The listing builds one solid part. Answer for the finished solid, in the listing's coordinates (mm). Face numbers are marked on the shaded views. A direction names the side the tool comes from. Round coordinates to 2 decimals unless told otherwise and drop trailing zeros. Order: outer loops, then holes, each group sorted by start corner. A loop starts at its lowest first (then second) coordinate and runs counter-clockwise, first axis right, second up. Notation, with made-up numbers: (72, -6.5) - (100, -6.5) arc R24 cw to (100, 13.5) - close; hole circle Ø8 at (33, -25.5). An arc over 180 degrees is marked (long way). Write item = value, one per line.
from build123d import *

# Parameters (mm, degrees)
SKETCH1_R           = 5
BOSS_EXTRUDE1_DEPTH = 25
SKETCH2_R           = 4
BOSS_EXTRUDE2_DEPTH = 20
SKETCH3_OUTSIDE_W   = 21.434
SKETCH3_OUTSIDE_H   = 21.434
SKETCH3_OUTSIDE_R   = 3
CUT_EXTRUDE1_DEPTH  = 2


with BuildPart() as part:
    # Sketch1 → Boss-Extrude1 (new body)
    with BuildSketch(Plane.XY):
        Circle(SKETCH1_R)
    extrude(amount=BOSS_EXTRUDE1_DEPTH)

    # Sketch2 → Boss-Extrude2 (add)
    with BuildSketch(Plane.XY.offset(25)):
        Circle(SKETCH2_R)
    extrude(amount=BOSS_EXTRUDE2_DEPTH)

    # Sketch3 outside → Cut-Extrude1 (cut)
    with BuildSketch(Plane.XY.offset(25)):
        Rectangle(SKETCH3_OUTSIDE_W, SKETCH3_OUTSIDE_H)
        Circle(SKETCH3_OUTSIDE_R, mode=Mode.SUBTRACT)
    extrude(amount=CUT_EXTRUDE1_DEPTH, mode=Mode.SUBTRACT)


solid = part.part
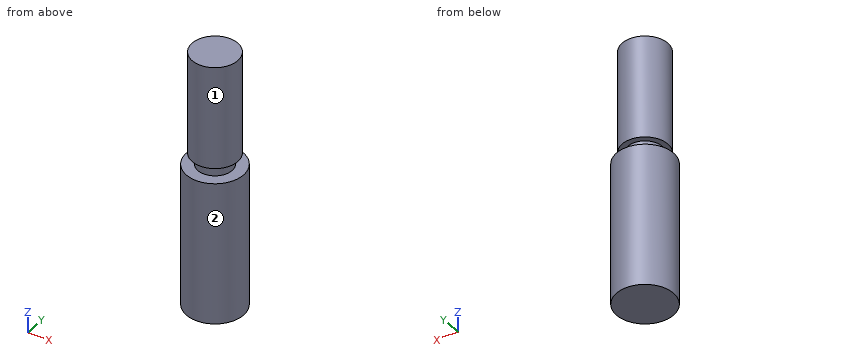
Q1. Section D-D on z = 22 is taken. Determine the outline of the cut face in (x, y), then the cut area to 3 significant figures.
Model answer:
outline = circle Ø10 at (0, 0)
area = 78.5 mm^2
Q2. For the marked faces 1 and 2, determine the directions among +Z, -Z, +X, -X, +Y, -Y from which every point of the face is accessible in a straight line to the end or side of a thin tool.
Model answer:
face_1 = +Z
face_2 = +Z, -Z
Q3. Find the intervals of material crossed by line 1 (Z direction, x = 0.5, y = 3); line 2 (X direction, y = -3, z = 18); line 3 (Y direction, x = -0.25, z = 20), in increasing order. Write a range as from..to.
Model answer:
line_1 = 0..25, 27..45
line_2 = -4..4
line_3 = -4.99..4.99
Q4. Section A-A on x = 0 is taken. Determine the outline of the cut face in (y, z), then the cut area to 3 significant figures.
Model answer:
outline = (-5, 0) - (5, 0) - (5, 25) - (3, 25) - (3, 27) - (4, 27) - (4, 45) - (-4, 45) - (-4, 27) - (-3, 27) - (-3, 25) - (-5, 25) - close
area = 406 mm^2
Q5. Section C-C on z = 37 is taken. Determine the outline of the cut face in (x, y), then the cut area to 3 significant figures.
Model answer:
outline = circle Ø8 at (0, 0)
area = 50.3 mm^2
Q6. Flat-ended cylindrical pins translate along their axes: P1, Ø5, axis at x = -3.5, z = 7.5, coming from the +Y side; P2, Ø1, axis at y = 2, z = 21, coming from the -X side; P3, Ø1.5, axis at y = 0.5, z = 6, coming from the -X side; P4, Ø5, axis at y = 2.5, z = 35.5, coming from the -X side. Find the tip coordinate at first contact, or state that the pin passes through.
Model answer:
P1 = 4.9
P2 = -4.77
P3 = -5
P4 = -4
